Design review of the part shown in the three views and the two pictorial views. Dimensions are in mm from the part's minimum x, y and z. A direction names the side the tool comes from. Round coordinates to 2 decimals unless told otherwise and drop trailing zeros. Order: outer loops, then holes, each group sorted by start corner. A loop starts at its lowest first (then second) coordinate and runs counter-clockwise, first axis right, second up. Notation, with made-up numbers: (40, -33.5) - (79, -33.5) arc R13 ccw to (79, -12.5) - close; hole circle Ø8 at (6.25, 17.25). An arc over 180 degrees is marked (long way). One line per question, with ' | ' between items. Start each with the question number.
Item 1: Add section A-A on y = 14. State the section outline as (x, z) points.
Item 2: Add section C-C on x = 16. State the section outline as (y, z) points, and give its area (3 significant figures).
Item 3: Draft analysis for pull direction Y (two halves, no side actions). For the marked faces 5, 6 and 7, state which applies: +Y half, -Y half, draft (parallel to the pull), parting line (faces both ways), or undercut.
Item 4: Add section B-B on z = 13. State the section outline as (x, y) points.
Item 5: Tool access review of the marked faces 1, 2, 3 and 4: name each direction out of +Z, -Z, +X, -X, +Y, -Y from which nothing blocks a thin tool from reaching the whole face with its end or side.
Item 6: Add section D-D on x = 5.25. State the section outline as (y, z) points.
Item 7: Insertion check: pin 1 Ø4 at (x, z) = (6, 27) entering from +Y; pin 2 Ø2 at (y, z) = (22, 5.5) entering from -X; pin 3 Ø12 at (x, z) = (5.5, 32.5) entering from -Y; pin 4 Ø3 at (x, y) = (18.5, 17) entering from +Z. Each pin has a flat end and moves straight along its axis. Give the tip position at first contact, or say it passes through.
Item 8: For L1, parallel to Y at x = 14, z = 19.5; L2, parallel to Z at x = 15.75, y = 23.5; L3, parallel to X at y = 20, z = 32.5 (1 decimal), list the stretches that pass through material, from the lowest coordinate up. Write a range as [from, to].
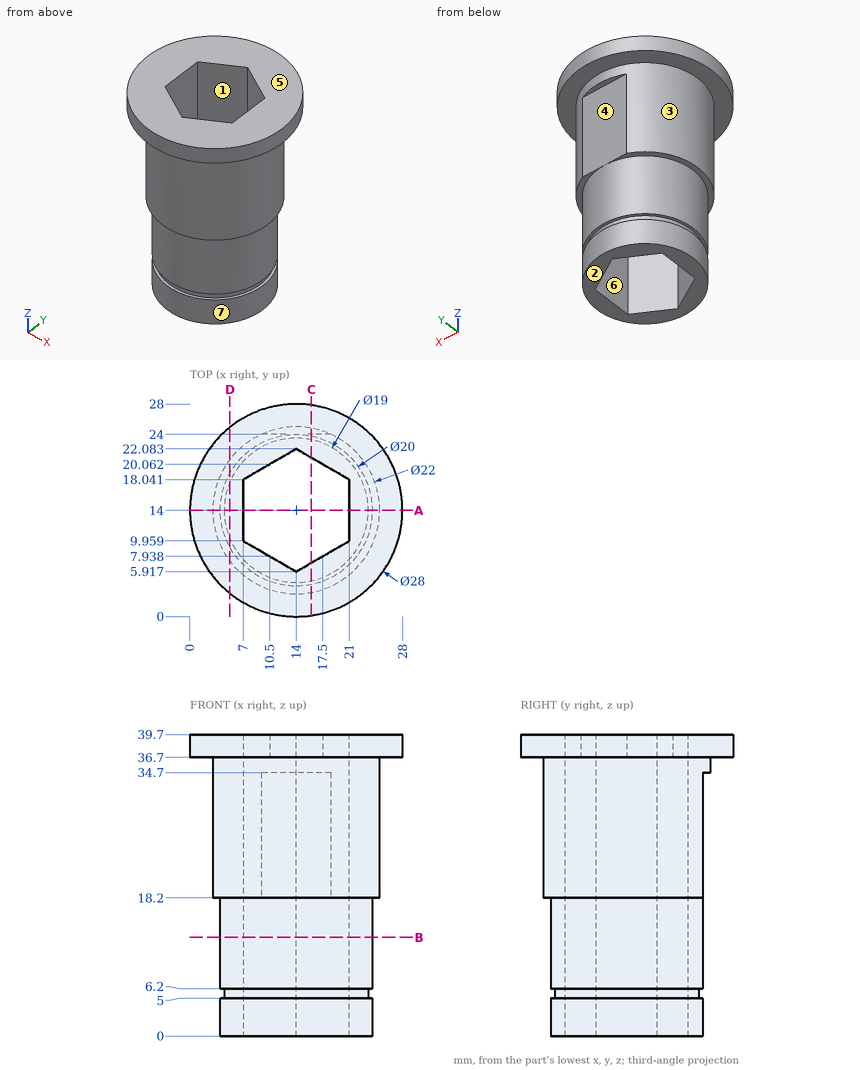
Determined:
1) outline: (0, 36.7) - (3, 36.7) - (3, 18.2) - (4, 18.2) - (4, 6.2) - (4.5, 6.2) - (4.5, 5) - (4, 5) - (4, 0) - (7, 0) - (7, 39.7) - (0, 39.7) - close; (21, 0) - (24, 0) - (24, 5) - (23.5, 5) - (23.5, 6.2) - (24, 6.2) - (24, 18.2) - (25, 18.2) - (25, 36.7) - (28, 36.7) - (28, 39.7) - (21, 39.7) - close
2) outline: (0.14, 36.7) - (3.18, 36.7) - (3.18, 18.2) - (4.2, 18.2) - (4.2, 6.2) - (4.71, 6.2) - (4.71, 5) - (4.2, 5) - (4.2, 0) - (7.07, 0) - (7.07, 39.7) - (0.14, 39.7) - close; (20.93, 0) - (23.8, 0) - (23.8, 5) - (23.29, 5) - (23.29, 6.2) - (23.8, 6.2) - (23.8, 18.2) - (24, 18.2) - (24, 34.7) - (24.82, 34.7) - (24.82, 36.7) - (27.86, 36.7) - (27.86, 39.7) - (20.93, 39.7) - close | area: 275 mm2
3) face 5: draft | face 6: undercut | face 7: parting line
4) outline: circle Ø20 at (14, 14); hole (7, 9.96) - (14, 5.92) - (21, 9.96) - (21, 18.04) - (14, 22.08) - (7, 18.04) - close
5) face 1: +Z, -Z | face 2: -Z, +X, -X, +Y, -Y | face 3: -Z | face 4: -Z, +X, -X, +Y
6) outline: (3.07, 36.7) - (7.33, 36.7) - (7.33, 18.2) - (9.16, 18.2) - (9.16, 6.2) - (10.3, 6.2) - (10.3, 5) - (9.16, 5) - (9.16, 0) - (18.84, 0) - (18.84, 5) - (17.7, 5) - (17.7, 6.2) - (18.84, 6.2) - (18.84, 18.2) - (20.67, 18.2) - (20.67, 36.7) - (24.93, 36.7) - (24.93, 39.7) - (3.07, 39.7) - close
7) pin 1: y = 23.22 | pin 2: x = 6.99 | pin 3: y = 0.65 | pin 4: through
8) L1: [3, 5.92], [22.08, 24] | L2: [0, 5], [6.2, 39.7] | L3: [4.8, 10.4], [17.6, 23.2]
